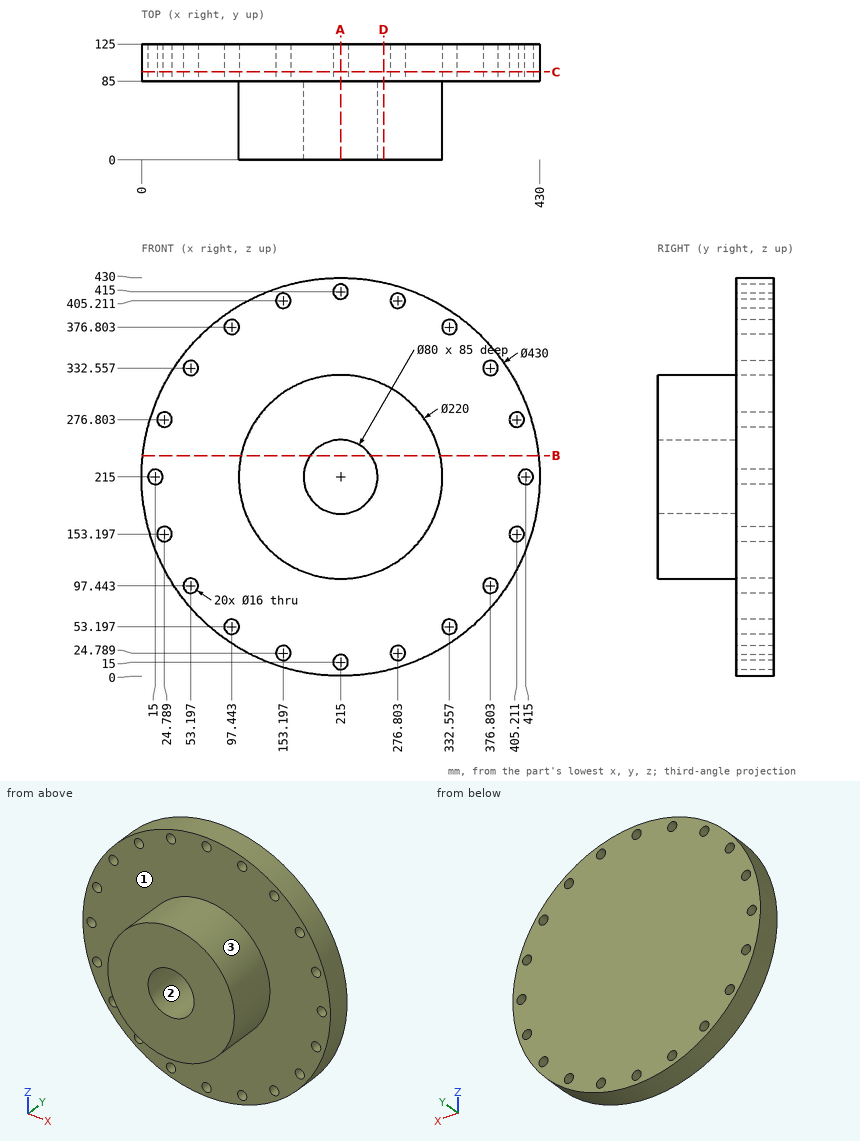
Design review of the part shown in the three views and the two pictorial views. Dimensions are in mm from the part's minimum x, y and z. Round coordinates to 2 decimals unless told otherwise and drop trailing zeros. Write each loop counter-clockwise with the first axis right and the second up, starting at its lowest first coordinate (ties: lowest second). Pieces come first, ordered by that corner, then holes. Notation, with made-up numbers: (-40, 8.5) - (-20, 8.5) arc R21 ccw to (-20, 36.5) - close; hole circle Ø11 at (29.25, 45). An arc over 180 degrees is marked (long way). Return JSON: item names as keys, results as strings. Group by question number.
Item 1: We need section D-D on x = 261.5. Write out the cut boundary in (y, z).
Item 2: The part is to be moulded in two halves that separate along X. For the marked faces 1, 2 and 3, say which applies: pulls with the +X half, pulls with the -X half, needs draft (parallel to the pull), parting line crosses it, or undercut.
Item 3: Insertion check: P1, Ø2, axis at x = 177, y = 28, coming from the -Z side; P2, Ø1.5, axis at x = 159.5, z = 129, coming from the -Y side; P3, Ø18.5, axis at x = 153.2, z = 24.79, coming from the -Y side; P4, Ø10, axis at y = 45.5, z = 126, coming from the +X side. Each pin has a flat end and moves straight along its axis. Give the tip position at first contact, or say it passes through.
Item 4: We need section C-C on y = 95. Give the number of separate pieces and of enclosed holes in the cut face, and give its area (3 significant figures).
Item 5: We need section A-A on x = 215. Write out the cut boundary in (y, z).
Item 6: For probe 1 along X at (y, z) = (108, 215); probe 2 along Z at (x, y) = (371.5, 94) (1 decimal); probe 3 along Y at (x, z) = (137, 339), list the stretches that pass through material, from the lowest coordinate up. Write a range as [from, to].
Item 7: We need section B-B on z = 238. Write out the cut boundary in (x, y), and give its area (3 significant figures).
Model answer:
{
 "1": {"outline": "(0, 115.31) - (85, 115.31) - (85, 5.09) - (125, 5.09) - (125, 424.91) - (85, 424.91) - (85, 314.69) - (0, 314.69) - close"},
 "2": {"face 1": "needs draft", "face 2": "undercut", "face 3": "parting line crosses it"},
 "3": {"P1": "stops at z = 111.41", "P2": "stops at y = 0", "P3": "stops at y = 85", "P4": "stops at x = 286.02"},
 "4": {"separate pieces": "1", "enclosed holes": "20", "area": "141,000 mm²"},
 "5": {"outline": "(0, 105) - (85, 105) - (85, 23) - (125, 23) - (125, 407) - (85, 407) - (85, 325) - (0, 325) - (0, 255) - (85, 255) - (85, 175) - (0, 175) - close; (85, 0) - (125, 0) - (125, 7) - (85, 7) - close; (85, 423) - (125, 423) - (125, 430) - (85, 430) - close"},
 "6": {"probe 1": "x = [0, 7], [23, 407], [423, 430]", "probe 2": "z = [67.6, 91.5], [103.4, 326.6], [338.5, 362.4]", "probe 3": "y = [85, 125]"},
 "7": {"outline": "(1.23, 85) - (107.43, 85) - (107.43, 0) - (182.27, 0) - (182.27, 85) - (247.73, 85) - (247.73, 0) - (322.57, 0) - (322.57, 85) - (428.77, 85) - (428.77, 125) - (1.23, 125) - close", "area": "29,800 mm²"}
}
